from build123d import *

# Parameters (mm, degrees)
SKETCH_1_R           = 2
SKETCH_1_R_2         = 0.75
BOSS_EXTRUDE_1_DEPTH = 1.5


with BuildPart() as part:
    # Sketch 1 → Boss-Extrude 1 (new body)
    with BuildSketch(Plane.XY):
        with BuildLine():
            Line((-57.299329586, 5), (6.700670414, 5))
            ThreePointArc((6.700670414, 5), (11.700670414, 0), (6.700670414, -5))
            Line((6.700670414, -5), (-57.299329586, -5))
            ThreePointArc((-57.299329586, -5), (-62.299329586, 0), (-57.299329586, 5))
        make_face()
        with Locations((-57.299329586, 0)):
            Circle(SKETCH_1_R, mode=Mode.SUBTRACT)
        with Locations((6.700670414, 0)):
            Circle(SKETCH_1_R_2, mode=Mode.SUBTRACT)
        with Locations((-41.299329586, 0)):
            Circle(SKETCH_1_R_2, mode=Mode.SUBTRACT)
        with Locations((-25.299329586, 0)):
            Circle(SKETCH_1_R, mode=Mode.SUBTRACT)
    extrude(amount=BOSS_EXTRUDE_1_DEPTH)


solid = part.part
Read the model definition and answer for the solid it produces. Units are mm, in the model's axes. Give positions to 0.01 mm unless a question says otherwise; leave off trailing zeros. Loops run counter-clockwise (first coordinate to the right, second up) from the corner with the lowest first, then second, coordinate; pieces in that order, holes last. Notation, with made-up numbers: (72, 2.5) -> (79, 2.5) arc R30 ccw to (79, 24.5) -> close; hole circle Ø11 at (-24, -2.5). An arc over 180 degrees is marked (long way). Use a Markdown table: item, result.
Q1. This flat-tipped pin is pushed along its axis until it touches: pin 1 (1.2 mm diameter, centred on x = -41.3, y = 0, fed in from -Z). Where does it stop, or does it pass through?
Solved:
| item | result |
|---|---|
| pin 1 | passes through |
Q2. Find the intervals of material crossed by line 1 along Y through (x, z) = (-25.5, 1.3); line 2 along X through (y, z) = (1.5, 0.2); line 3 along X through (y, z) = (-0.5, 0.65), in increasing order.
Solved:
| item | result |
|---|---|
| line 1 | y = -5 to -1.99, 1.99 to 5 |
| line 2 | x = -62.07 to -58.62, -55.98 to -26.62, -23.98 to 11.47 |
| line 3 | x = -62.27 to -59.24, -55.36 to -41.86, -40.74 to -27.24, -23.36 to 6.14, 7.26 to 11.68 |
Q3. Section B-B, the plane z = 0.95 is taken. Determine the outline of the cut face in (x, y), then the cut area to 3 significant figures.
Solved:
| item | result |
|---|---|
| outline | (-57.3, -5) -> (6.7, -5) arc R5 ccw to (6.7, 5) -> (-57.3, 5) arc R5 ccw to start; hole circle Ø4 at (-57.3, 0); hole circle Ø1.5 at (-41.3, 0); hole circle Ø4 at (-25.3, 0); hole circle Ø1.5 at (6.7, 0) |
| area | 690 mm^2 |
Q4. Section A-A, the plane y = 0 is taken. Determine the outline of the cut face in (x, z), then the cut area to 3 significant figures.
Solved:
| item | result |
|---|---|
| outline | (-62.3, 0) -> (-59.3, 0) -> (-59.3, 1.5) -> (-62.3, 1.5) -> close; (-55.3, 0) -> (-42.05, 0) -> (-42.05, 1.5) -> (-55.3, 1.5) -> close; (-40.55, 0) -> (-27.3, 0) -> (-27.3, 1.5) -> (-40.55, 1.5) -> close; (-23.3, 0) -> (5.95, 0) -> (5.95, 1.5) -> (-23.3, 1.5) -> close; (7.45, 0) -> (11.7, 0) -> (11.7, 1.5) -> (7.45, 1.5) -> close |
| area | 94.5 mm^2 |
Q5. Section C-C, the plane y = -3.75 is taken. Determine the outline of the cut face in (x, z), then the cut area to 3 significant figures.
Solved:
| item | result |
|---|---|
| outline | (-60.61, 0) -> (10.01, 0) -> (10.01, 1.5) -> (-60.61, 1.5) -> close |
| area | 106 mm^2 |
Q6. Determine the mould class of faces 1 (the face through (-62.3, -0.1, 0.7)), 2 (the face through (-25, -5, 1)), 3 (the face through (-23.39, 0.6, 0.74)) for opening direction Y: pulls with the +Y half, pulls with the -Y half, needs draft (parallel to the pull), parting line crosses it, or undercut.
Solved:
| item | result |
|---|---|
| face 1 | parting line crosses it |
| face 2 | pulls with the -Y half |
| face 3 | undercut |
